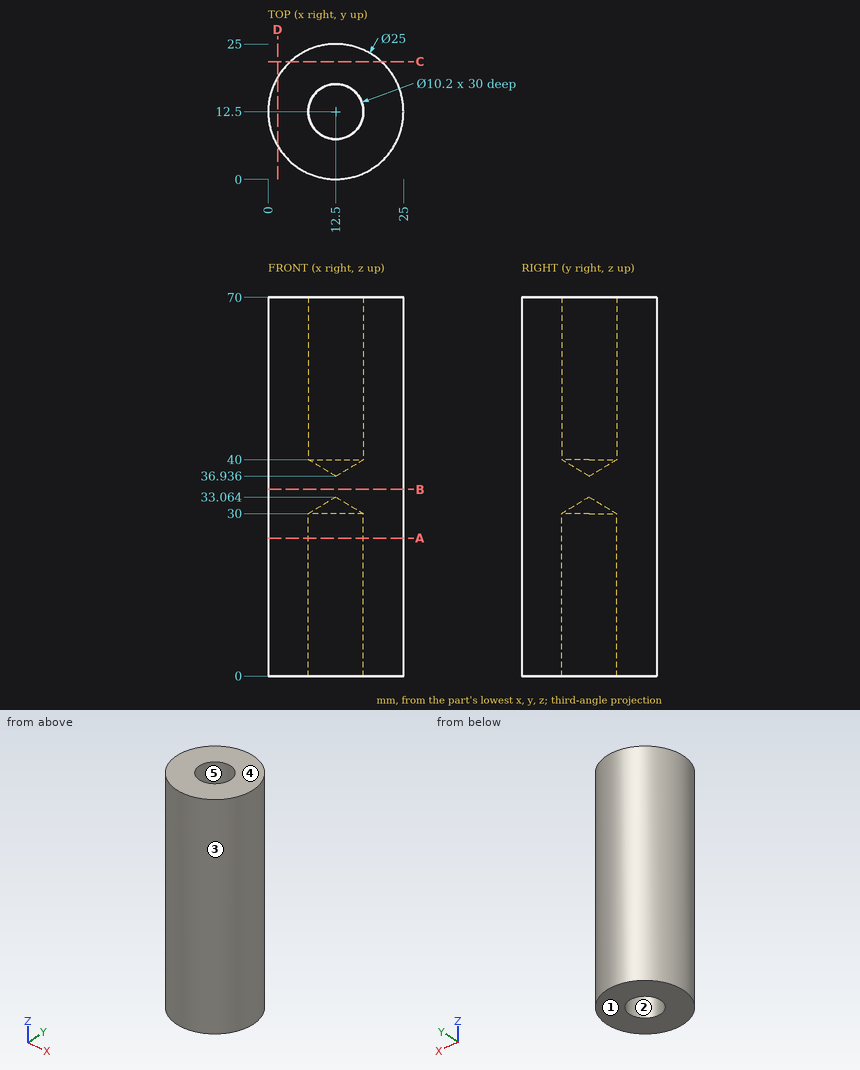
For this review, use the dimensioned drawing (mm, ordinates from the lowest corner) and the shaded views. A direction names the side the tool comes from. Round coordinates to 2 decimals unless told otherwise and drop trailing zeros. Order: outer loops, then holes, each group sorted by start corner. A loop starts at its lowest first (then second) coordinate and runs counter-clockwise, first axis right, second up. Notation, with made-up numbers: M 24,-26 L 79,-26 A24 ccw 79,0 Z; hole C 61.25,9.5 d6. An arc over 180 degrees is marked long. Use a Markdown table: item, result.
1) Consider section B-B (z = 34.5). Write out the cut boundary in (x, y).
Report:
| item | result |
|---|---|
| outline | C 12.5,12.5 d25 |
2) Wall thickness on line 1 along Y through (x, z) = (12.5, 47.25); line 2 along X through (y, z) = (16, 16): over which ranges is each line inside the solid? List them lowest first. Write a range as [from, to].
Report:
| item | result |
|---|---|
| line 1 | [0, 7.4], [17.6, 25] |
| line 2 | [0.5, 8.79], [16.21, 24.5] |
3) Draft analysis for pull direction X (two halves, no side actions). For the marked faces 1, 2 and 3, state which applies: released by +X, released by -X, zero draft, split by the parting line, or undercut.
Report:
| item | result |
|---|---|
| face 1 | zero draft |
| face 2 | undercut |
| face 3 | split by the parting line |
4) Insertion check: pin 1 (12 mm diameter, centred on y = 20.5, z = 57.5, fed in from -X); pin 2 (6 mm diameter, centred on x = 10.5, z = 60.5, fed in from +Y); pin 3 (1.5 mm diameter, centred on y = 7.5, z = 31, fed in from +X) (1 decimal); pin 4 (2 mm diameter, centred on y = 20, z = 37.5, fed in from -X). Each pin has a flat end and moves straight along its axis. Give the tip position at first contact, or say it passes through.
Report:
| item | result |
|---|---|
| pin 1 | x = 0.16 |
| pin 2 | y = 25 |
| pin 3 | x = 24.3 |
| pin 4 | x = 1.82 |
5) Tool access review of the marked faces 4 and 5: name each direction out of +Z, -Z, +X, -X, +Y, -Y from which nothing blocks a thin tool from reaching the whole face with its end or side.
Report:
| item | result |
|---|---|
| face 4 | +Z, +X, -X, +Y, -Y |
| face 5 | +Z |
6) Consider section D-D (x = 1.75). Write out the cut boundary in (y, z).
Report:
| item | result |
|---|---|
| outline | M 6.12,0 L 18.88,0 L 18.88,70 L 6.12,70 Z |
7) Consider section A-A (z = 25.5). Write out the cut boundary in (x, y), then the cut area to 3 significant figures.
Report:
| item | result |
|---|---|
| outline | C 12.5,12.5 d25; hole C 12.5,12.5 d10.2 |
| area | 409 mm^2 |
8) Consider section C-C (y = 21.75). Write out the cut boundary in (x, z).
Report:
| item | result |
|---|---|
| outline | M 4.09,0 L 20.91,0 L 20.91,70 L 4.09,70 Z |
